Can you work these out from the model? Positions are in its coordinate system, mm. Coordinates: 2 decimals unless noted, no trailing zeros. Order: outer loops, then holes, each group sorted by start corner. A loop starts at its lowest first (then second) coordinate and runs counter-clockwise, first axis right, second up.
```python
from build123d import *

# Parameters (mm, degrees)
EXTRUDE_1_DEPTH = 1145


with BuildPart() as part:
    # 草图2 → 凸台-拉伸1 (new, symmetric)
    with BuildSketch(Plane.XY):
        with BuildLine():
            Line((-11.25, 5.782842712), (-10.667157288, 5.199999999))
            Line((-10.667157288, 5.199999999), (-8.25, 5.199999999))
            Line((-8.25, 5.199999999), (-8.25, 6))
            Line((-8.25, 6), (-10.25, 6))
            Line((-10.25, 6), (-10.25, 7.726142057))
            Line((-10.25, 7.726142057), (-8.999999375, 7.724528349))
            Line((-8.999999375, 7.724528349), (-8.25, 8.473560125))
            Line((-8.25, 8.473560125), (-8.25, 8.88650173))
            ThreePointArc((-8.25, 8.88650173), (-5.642322013, 8.341793831), (-3, 8.002934636))
            Line((-3, 8.002934636), (-3, 7.70225919))
            Line((-3, 7.70225919), (3, 7.70225919))
            Line((3, 7.70225919), (3, 8.002934636))
            ThreePointArc((3, 8.002934636), (5.642322013, 8.341793831), (8.25, 8.88650173))
            Line((8.25, 8.88650173), (8.25, 8.473560125))
            Line((8.25, 8.473560125), (8.999999375, 7.724528349))
            Line((8.999999375, 7.724528349), (10.25, 7.726142057))
            Line((10.25, 7.726142057), (10.25, 6))
            Line((10.25, 6), (8.25, 6))
            Line((8.25, 6), (8.25, 5.2))
            Line((8.25, 5.2), (10.667157288, 5.2))
            Line((10.667157288, 5.2), (11.25, 5.782842712))
            Line((11.25, 5.782842712), (11.25, 9.785632758))
            ThreePointArc((11.25, 9.785632758), (17.712457567, 12.84892987), (23.391097866, 17.196364903))
            Line((23.391097866, 17.196364903), (23.391097866, 18.63499481))
            ThreePointArc((23.391097866, 18.63499481), (23.329308001, 18.727406852), (23.220298155, 18.705616343))
            ThreePointArc((23.220298155, 18.705616343), (0, 9.070311977), (-23.220298155, 18.705616342))
            ThreePointArc((-23.220298155, 18.705616342), (-23.329308002, 18.727406852), (-23.391097866, 18.634994809))
            Line((-23.391097866, 18.634994809), (-23.391097866, 17.196364902))
            ThreePointArc((-23.391097866, 17.196364902), (-17.712457568, 12.84892987), (-11.25, 9.785632758))
            Line((-11.25, 9.785632758), (-11.25, 5.782842712))
        make_face()
    extrude(amount=EXTRUDE_1_DEPTH, both=True)


solid = part.part
```
1. I'm going to push flat-ended pins straight in: pin 1 (4 mm diameter, centred on y = 12.5, z = -321.5, fed in from +X); pin 2 (1 mm diameter, centred on x = 9, z = -405.5, fed in from +Y); pin 3 (3 mm diameter, centred on x = -1.5, z = 304, fed in from -Y). Where does each tip first touch, or does it pass through?
Completed:
pin 1: stops at x = 20.17
pin 2: stops at y = 10.48
pin 3: stops at y = 7.7
2. Imagine slicing it at A-A on y = 14.5. Please give me the cut outline in (x, z).
Completed:
outline: (-20.17, -1145) - (-18.07, -1145) - (-18.07, 1145) - (-20.17, 1145) - close; (18.07, -1145) - (20.17, -1145) - (20.17, 1145) - (18.07, 1145) - close
3. Please list where these lines run through material, in increasing order: probe 1 along X at (y, z) = (6.25, 49); probe 2 along Y at (x, z) = (-10, 899.5); probe 3 along Y at (x, z) = (2.5, 788).
Completed:
probe 1: x = -11.25 to -10.25, 10.25 to 11.25
probe 2: y = 5.2 to 6, 7.73 to 10.63
probe 3: y = 7.7 to 9.17
